Could you check a few things on this model? Use its own coordinates, in mm. A direction names the side the tool comes from. Give positions to 0.01 mm unless a question says otherwise; leave off trailing zeros. Order: outer loops, then holes, each group sorted by start corner. A loop starts at its lowest first (then second) coordinate and runs counter-clockwise, first axis right, second up.
from build123d import *

# Parameters (mm, degrees)
BASE_PLATE_SKETCH_W         = 50
BASE_PLATE_SKETCH_H         = 70
BASE_PLATE_DEPTH            = 9
U_FRAME_SKETCH_W            = 16
U_FRAME_SKETCH_H            = 11
U_FRAME_DEPTH               = 70
SIDE_BLOCK_A_SKETCH_W       = 34
SIDE_BLOCK_A_SKETCH_H       = 50
SIDE_BLOCK_A_DEPTH          = 16
SIDE_BLOCK_B_SKETCH_W       = 34
SIDE_BLOCK_B_SKETCH_H       = 50
SIDE_BLOCK_B_DEPTH          = 16
BASE_RECESS_SKETCH_W        = 50
BASE_RECESS_SKETCH_H        = 70
BASE_RECESS_CUT_DEPTH       = 3
TOP_LIP_SKETCH_W            = 16
TOP_LIP_SKETCH_H            = 20
TOP_LIP_DEPTH               = 3
CYLINDER_SKETCH_R           = 25
CYLINDER_50_DEPTH           = 70
CYLINDER_START              = 20
CYLINDER_EXTENSION_SKETCH_R = 25
CYLINDER_EXTENSION_50_DEPTH = 20
U_SLOT_CUT_DEPTH            = 60
FRAME_CLEARANCE_SKETCH_W    = 18
FRAME_CLEARANCE_SKETCH_H    = 21
FRAME_CLEARANCE_CUT_DEPTH   = 50
END_FLAT_A_DEPTH            = 10
END_START                   = -10
END_FLAT_B_DEPTH            = 10


with BuildPart() as part:
    # Base Plate Sketch → Base Plate (new body)
    with BuildSketch(Plane.XY):
        with Locations((25, -35)):
            Rectangle(BASE_PLATE_SKETCH_W, BASE_PLATE_SKETCH_H)
    extrude(amount=BASE_PLATE_DEPTH)

    # U-Frame Sketch → U-Frame (add)
    with BuildSketch(Plane.XZ.offset(70)):
        with Locations((8, 14.5)):
            Rectangle(U_FRAME_SKETCH_W, U_FRAME_SKETCH_H)
        with Locations((42, 14.5)):
            Rectangle(U_FRAME_SKETCH_W, U_FRAME_SKETCH_H)
    extrude(amount=-U_FRAME_DEPTH)

    # Side Block A Sketch → Side Block A (add)
    with BuildSketch(Plane.ZY):
        with Locations((37, -25)):
            Rectangle(SIDE_BLOCK_A_SKETCH_W, SIDE_BLOCK_A_SKETCH_H)
    extrude(amount=-SIDE_BLOCK_A_DEPTH)

    # Side Block B Sketch → Side Block B (add)
    with BuildSketch(Plane(origin=(50, 0, 0), x_dir=(0, 0, -1), z_dir=(1, 0, 0))):
        with Locations((-37, -25)):
            Rectangle(SIDE_BLOCK_B_SKETCH_W, SIDE_BLOCK_B_SKETCH_H)
    extrude(amount=-SIDE_BLOCK_B_DEPTH)

    # Base Recess Sketch → Base Recess Cut (cut)
    with BuildSketch(Plane(origin=(0, 0, 0), x_dir=(-1, 0, 0), z_dir=(0, 0, -1))):
        with Locations((-25, -35)):
            Rectangle(BASE_RECESS_SKETCH_W, BASE_RECESS_SKETCH_H)
    extrude(amount=-BASE_RECESS_CUT_DEPTH, mode=Mode.SUBTRACT)

    # Top Lip Sketch → Top Lip (add)
    with BuildSketch(Plane.XY.offset(20)):
        with Locations((8, -60)):
            Rectangle(TOP_LIP_SKETCH_W, TOP_LIP_SKETCH_H)
        with Locations((42, -60)):
            Rectangle(TOP_LIP_SKETCH_W, TOP_LIP_SKETCH_H)
    extrude(amount=TOP_LIP_DEPTH)

    # Cylinder Sketch → Cylinder Ø50 (add)
    with BuildSketch(Plane.ZY):
        with Locations((58, -35)):
            Circle(CYLINDER_SKETCH_R)
    extrude(amount=-CYLINDER_50_DEPTH)

    # Cylinder Extension Sketch → Cylinder Extension Ø50 (add)
    with BuildSketch(Plane.ZY.offset(CYLINDER_START)):
        with Locations((58, -35)):
            Circle(CYLINDER_EXTENSION_SKETCH_R)
    extrude(amount=-CYLINDER_EXTENSION_50_DEPTH)

    # U-Slot Sketch → U-Slot Cut (cut)
    with BuildSketch(Plane.XY.offset(23)):
        Polygon((34, -70), (50, -70), (50, -50), (0, -50), (0, -70), align=None)
    extrude(amount=U_SLOT_CUT_DEPTH, mode=Mode.SUBTRACT)

    # Frame Clearance Sketch → Frame Clearance Cut (cut)
    with BuildSketch(Plane.XZ.offset(50)):
        with Locations((25, 43.5)):
            Rectangle(FRAME_CLEARANCE_SKETCH_W, FRAME_CLEARANCE_SKETCH_H)
    extrude(amount=-FRAME_CLEARANCE_CUT_DEPTH, mode=Mode.SUBTRACT)

    # End Flat A Sketch → End Flat A (cut)
    with BuildSketch(Plane.ZY.offset(20)):
        with BuildLine():
            Line((71, -13.645843496), (71, -56.354156504))
            ThreePointArc((71, -56.354156504), (83, -35), (71, -13.645843496))
        make_face()
    extrude(amount=-END_FLAT_A_DEPTH, mode=Mode.SUBTRACT)

    # End Flat B Sketch → End Flat B (cut)
    with BuildSketch(Plane(origin=(70, 0, 0), x_dir=(0, 0, -1), z_dir=(1, 0, 0)).offset(END_START)):
        with BuildLine():
            Line((-71, -13.645843496), (-71, -56.354156504))
            ThreePointArc((-71, -56.354156504), (-83, -35), (-71, -13.645843496))
        make_face()
    extrude(amount=END_FLAT_B_DEPTH, mode=Mode.SUBTRACT)


solid = part.part
Item 1: Please list where these lines run through material, in increasing order: line 1 along X through (y, z) = (-15.5, 37); line 2 along Z through (x, y) = (26.5, -35); line 3 along Z through (x, y) = (27, -20).
Findings:
line 1: x = 0 to 16, 34 to 50
line 2: z = 3 to 9, 54 to 83
line 3: z = 3 to 9, 54 to 78
Item 2: For pin 1 (3 mm diameter, centred on x = 40, y = -3, fed in from +Z); pin 2 (12 mm diameter, centred on x = -8.5, z = 37, fed in from -Y); pin 3 (13 mm diameter, centred on x = 38.5, y = -57, fed in from +Z); pin 4 (6 mm diameter, centred on x = 28.5, z = 29, fed in from -Y), each with a flat end and sliding along its axis, tell me the tip position at first contact or that it passes through.
Findings:
pin 1: stops at z = 54
pin 2: stops at y = -55
pin 3: stops at z = 23
pin 4: passes through
Item 3: For faces 5 (the flat face through (-15, -35, 71)), 6 (the flat face through (50, -54, 58)), 7 (the flat face through (60, -35, 76)), 8 (the flat face through (25, -35, 9)), which set-ups out of +Z, -Z, +X, -X, +Y, -Y let a thin tool reach every point of the face, with its end or its side?
Findings:
face 5: +Z, -X, +Y, -Y
face 6: +Z, -Y
face 7: +Z, +X, +Y, -Y
face 8: +Y, -Y
Item 4: Imagine slicing it at C-C on z = 16. List the corners of the cut face in (x, y) for me, then the cut area to 3 significant figures.
Findings:
outline: (0, -70) - (16, -70) - (16, 0) - (0, 0) - close; (34, -70) - (50, -70) - (50, 0) - (34, 0) - close
area: 2,240 mm2
Item 5: Imagine slicing it at B-B on y = -35. List the corners of the cut face in (x, z) for me.
Findings:
outline: (-20, 33) - (0, 33) - (0, 3) - (50, 3) - (50, 33) - (70, 33) - (70, 71) - (60, 71) - (60, 83) - (-10, 83) - (-10, 71) - (-20, 71) - close; hole (16, 9) - (34, 9) - (34, 54) - (16, 54) - close
Item 6: Imagine slicing it at D-D on z = 58. List the corners of the cut face in (x, y) for me.
Findings:
outline: (-20, -60) - (0, -60) - (0, -50) - (50, -50) - (50, -60) - (70, -60) - (70, -10) - (-20, -10) - close
Item 7: Imagine slicing it at A-A on x = 20.5. List the corners of the cut face in (y, z) for me.
Findings:
outline: (-70, 3) - (0, 3) - (0, 9) - (-70, 9) - close; (-50, 54) - (-10.32, 54) arc R25 ccw to (-50, 78) - close
Item 8: We'd pull the mould along X, two halves only. Please class faces 1 (the flat face through (-10, -35, 76)), 2 (the flat face through (25, -30, 54)), 3 (the flat face through (50, -27, 23)), 4 (the flat face through (0, -54, 58)): +X half, -X half, draft (parallel to the pull), parting line (faces both ways), or undercut.
Findings:
face 1: -X half
face 2: undercut
face 3: +X half
face 4: undercut
